Here's how the part is built. I have some questions about the finished solid (model axes, mm). Face numbers are marked on the shaded views. Round coordinates to 2 decimals unless told otherwise and drop trailing zeros. Write each loop counter-clockwise with the first axis right and the second up, starting at its lowest first coordinate (ties: lowest second). Pieces come first, ordered by that corner, then holes. Notation, with made-up numbers: (-37.5, -39.75) - (16.5, -39.75) arc R8 ccw to (16.5, -30.75) - close; hole circle Ø11 at (13.25, 14.25). An arc over 180 degrees is marked (long way). One line per question, with ' | ' between items. Start each with the question number.
(1) Imagine slicing it at B-B (y = 1). Write out the boundary of the cut face in (x, z).
(2) Imagine slicing it at A-A (z = 0). Write out the boundary of the cut face in (x, y), plus the area to 3 significant figures.
(3) Imagine slicing it at C-C (y = -6.5). Write out the boundary of the cut face in (x, z).
(4) Thinking about a two-plate mould opening in X: for the marked faces 1 and 2, which applies, pulls with the +X half, pulls with the -X half, needs draft (parallel to the pull), parting line crosses it, or undercut?
(5) Imagine slicing it at D-D (z = 22.5). Give the number of separate pieces and of enclosed holes in the cut face, plus the area to 3 significant figures.
(6) If I drill on L1, parallel to X at y = 1.25, z = -26.5; L2, parallel to X at y = -2.25, z = 2; L3, parallel to Y at x = -39, z = 11.5, over which ranges is the centre line in solid material (lowest first)?
(7) Will these pins go through, and if not, where does the flat tip stop? pin 1 (12 mm diameter, centred on x = 0, z = 0, fed in from -Y); pin 2 (2 mm diameter, centred on y = -7, z = -20.5, fed in from +X); pin 3 (8 mm diameter, centred on x = -25.5, z = 25, fed in from -Y).
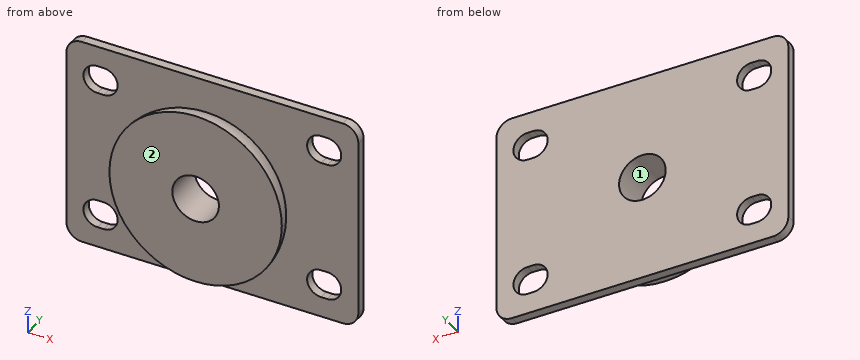
from build123d import *

# Parameters (mm, degrees)
SKETCH_2_W          = 94
SKETCH_2_H          = 67
EXTRUDE_1_DEPTH     = 3
FILLET_1_R          = 5
CUT_EXTRUDE_1_DEPTH = 58.794895968
SKETCH_6_R          = 7.5
CUT_EXTRUDE_2_DEPTH = 60.055059055


with BuildPart() as part:
    # 草图2 → 拉伸1 (new body)
    with BuildSketch(Plane(origin=(0, 0, 0), x_dir=(1, 0, 0), z_dir=(0, 1, 0))):
        Rectangle(SKETCH_2_W, SKETCH_2_H)
    extrude(amount=EXTRUDE_1_DEPTH)

    # 圆角1
    fillet_1_edges = [part.edges().sort_by_distance(p)[0] for p in [
        (-47, 1.5, -33.5),
        (47, 1.5, -33.5),
        (47, 1.5, 33.5),
        (-47, 1.5, 33.5),
    ]]
    fillet(fillet_1_edges, radius=FILLET_1_R)

    # 草图3 → 切除-拉伸1 (cut, through all)
    with BuildSketch(Plane(origin=(0, 3, 0), x_dir=(-1, 0, 0), z_dir=(0, 1, 0))):
        with BuildLine():
            Line((35, 27), (37, 27))
            ThreePointArc((37, 27), (41.5, 22.5), (37, 18))
            Line((37, 18), (35, 18))
            ThreePointArc((35, 18), (30.5, 22.5), (35, 27))
        make_face()
        with BuildLine():
            Line((-35, 18), (-37, 18))
            ThreePointArc((-37, 18), (-41.5, 22.5), (-37, 27))
            Line((-37, 27), (-35, 27))
            ThreePointArc((-35, 27), (-30.5, 22.5), (-35, 18))
        make_face()
        with BuildLine():
            Line((-35, -27), (-37, -27))
            ThreePointArc((-37, -27), (-41.5, -22.5), (-37, -18))
            Line((-37, -18), (-35, -18))
            ThreePointArc((-35, -18), (-30.5, -22.5), (-35, -27))
        make_face()
        with BuildLine():
            Line((35, -18), (37, -18))
            ThreePointArc((37, -18), (41.5, -22.5), (37, -27))
            Line((37, -27), (35, -27))
            ThreePointArc((35, -27), (30.5, -22.5), (35, -18))
        make_face()
    extrude(amount=-CUT_EXTRUDE_1_DEPTH, mode=Mode.SUBTRACT)

    # 草图4 → 旋转1 (revolve)
    with BuildSketch(Plane.XY, mode=Mode.PRIVATE) as revolve_1_sk:
        with BuildLine():
            Line((0, -9.5), (27.75, -9.5))
            ThreePointArc((27.75, -9.5), (24.967514421, -2.782485579), (18.25, 0))
            Line((18.25, 0), (0, 0))
            Line((0, 0), (0, -9.5))
        make_face()
    revolve(revolve_1_sk.sketch.rotate(Axis((0, 11.062770563, 0), (0, -1, 0)), 90), axis=Axis((0, 11.062770563, 0), (0, -1, 0)))

    # 草图6 → 切除-拉伸2 (cut, through all)
    with BuildSketch(Plane.XZ.offset(9.5)):
        with Locations(Location((0, 0, 0), (0, 0, 270))):
            Circle(SKETCH_6_R)
    extrude(amount=-CUT_EXTRUDE_2_DEPTH, mode=Mode.SUBTRACT)


solid = part.part
Check sheet entries:
1) outline: (-47, -28.5) arc R5 ccw to (-42, -33.5) - (42, -33.5) arc R5 ccw to (47, -28.5) - (47, 28.5) arc R5 ccw to (42, 33.5) - (-42, 33.5) arc R5 ccw to (-47, 28.5) - close; hole (-37, -27) - (-35, -27) arc R4.5 ccw to (-35, -18) - (-37, -18) arc R4.5 ccw to start; hole (-37, 18) - (-35, 18) arc R4.5 ccw to (-35, 27) - (-37, 27) arc R4.5 ccw to start; hole circle Ø15 at (0, 0); hole (35, -27) - (37, -27) arc R4.5 ccw to (37, -18) - (35, -18) arc R4.5 ccw to start; hole (35, 18) - (37, 18) arc R4.5 ccw to (37, 27) - (35, 27) arc R4.5 ccw to start
2) outline: (-47, 0) - (-18.25, 0) arc R9.5 ccw to (-27.75, -9.5) - (-7.5, -9.5) - (-7.5, 3) - (-47, 3) - close; (7.5, -9.5) - (27.75, -9.5) arc R9.5 ccw to (18.25, 0) - (47, 0) - (47, 3) - (7.5, 3) - close | area: 583 mm^2
3) outline: circle Ø54.53 at (0, 0); hole circle Ø15 at (0, 0)
4) face 1: undercut | face 2: needs draft
5) separate pieces: 4 | enclosed holes: 0 | area: 440 mm^2
6) L1: -47 to -39.06, -32.94 to 32.94, 39.06 to 47 | L2: -24.31 to -7.23, 7.23 to 24.31 | L3: 0 to 3
7) pin 1: through | pin 2: x = 19.33 | pin 3: y = 0
